Verification items for this drawing (mm, ordinates from the low corner). Give positions to 0.01 mm unless a question says otherwise; leave off trailing zeros. Loops run counter-clockwise (first coordinate to the right, second up) from the corner with the lowest first, then second, coordinate; pieces in that order, holes last. Notation, with made-up numbers: (-2, 59) -> (34, 59) arc R16 ccw to (34, 67) -> close; hole circle Ø2 at (69.5, 88.25). An arc over 180 degrees is marked (long way). Write item = value, one per line.
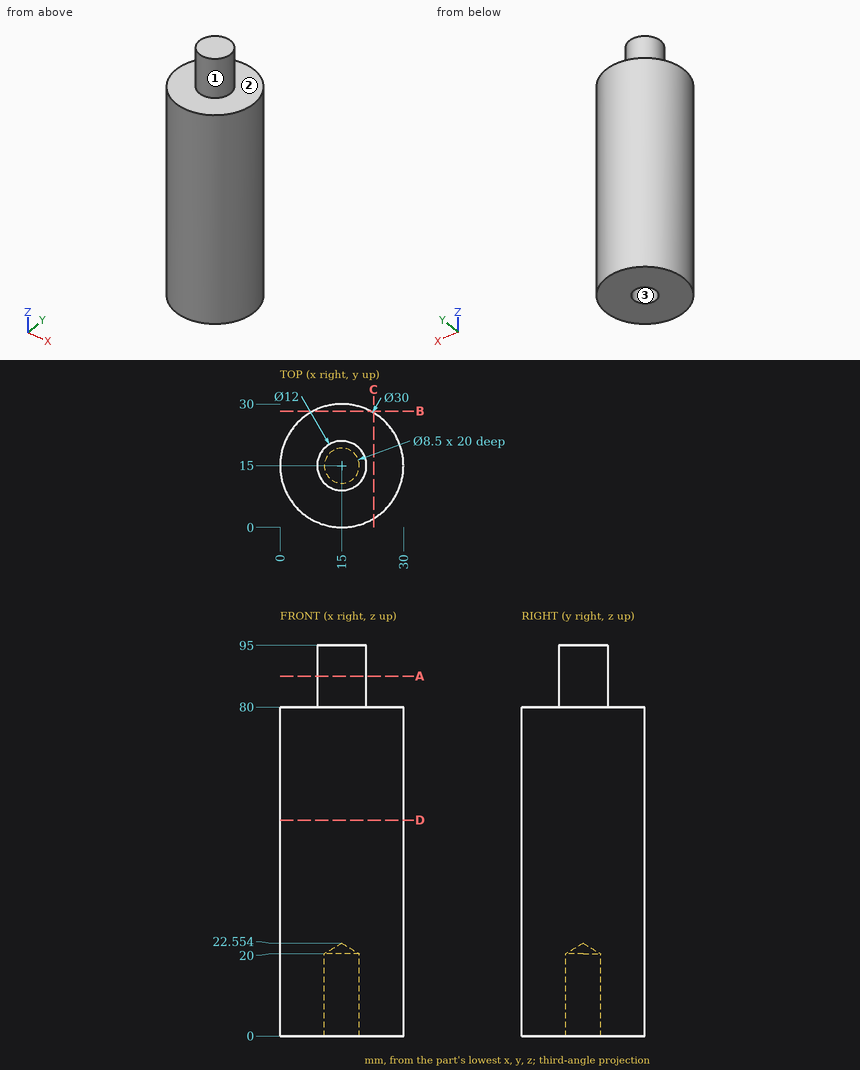
Item 1: Gauge pin test, flat ends, axial feed: pin 1 (5 mm diameter, centred on x = 7, z = 30, fed in from -Y) (1 decimal); pin 2 (10 mm diameter, centred on x = 3, z = 27, fed in from +Y); pin 3 (1 mm diameter, centred on x = 26.5, y = 23, fed in from +Z). Record the tip position at first contact, or that the pin passes through.
Answer:
pin_1 = 1
pin_2 = 28.27
pin_3 = 80
Item 2: Section check B-B, the plane y = 28.25. Record the cut outline in (x, z), plus the area to 4 significant figures.
Answer:
outline = (7.97, 0) -> (22.03, 0) -> (22.03, 80) -> (7.97, 80) -> close
area = 1,125 mm^2
Item 3: Thickness scan on L1, parallel to Y at x = 15, z = 14.5; L2, parallel to Z at x = 18, y = 6; L3, parallel to X at y = 11.75, z = 8.5 (1 decimal). Record the ranges inside material, lowest first. Write a range as [from, to].
Answer:
L1 = [0, 10.75], [19.25, 30]
L2 = [0, 80]
L3 = [0.4, 12.3], [17.7, 29.6]
Item 4: Section check C-C, the plane x = 22.75. Record the cut outline in (y, z), plus the area to 3 significant figures.
Answer:
outline = (2.16, 0) -> (27.84, 0) -> (27.84, 80) -> (2.16, 80) -> close
area = 2,050 mm^2
Item 5: Section check D-D, the plane z = 52.5. Record the cut outline in (x, y), plus the area to 3 significant figures.
Answer:
outline = circle Ø30 at (15, 15)
area = 707 mm^2
Item 6: Draft check along X on the marked faces 1, 2 and 3. Enter one of: +X half, -X half, draft (parallel to the pull), parting line (faces both ways), or undercut.
Answer:
face_1 = parting line
face_2 = draft
face_3 = undercut
Item 7: Section check A-A, the plane z = 87.5. Record the cut outline in (x, y).
Answer:
outline = circle Ø12 at (15, 15)
